Design review of the part built by this model. Coordinates are the model's own, in mm. Face numbers are marked on the shaded views. A direction names the side the tool comes from. Round coordinates to 2 decimals unless told otherwise and drop trailing zeros. Loops run counter-clockwise (first coordinate to the right, second up) from the corner with the lowest first, then second, coordinate; pieces in that order, holes last. Notation, with made-up numbers: (-26, 76) - (3, 76) arc R3 ccw to (3, 81) - close; hole circle Ø5 at (3, 60). An arc over 180 degrees is marked (long way). Use one line per item in the form item = value. Start each with the question number.
(1) We need section B-B, the plane z = 23. Write out the cut boundary in (x, y), then the cut area to 3 significant figures.
(2) Machinability: for the marked faces 1, 2 and 3, which of the approach directions +Z, -Z, +X, -X, +Y, -Y give a long, thin tool a straight path to every point of the face, cutting with its end or side? Answer none if there is none.
(3) We need section A-A, the plane z = 62.5. Write out the cut boundary in (x, y), then the cut area to 3 significant figures.
(4) We need section C-C, the plane z = 44. Write out the cut boundary in (x, y).
(5) For pin 1 (5.5 mm diameter, centred on x = -1, z = 48, fed in from -Y); pin 2 (2 mm diameter, centred on y = -5.5, z = 49.5, fed in from +X); pin 3 (3 mm diameter, centred on y = -5.5, z = 53, fed in from -X), all flat-tipped, find the tip position at first contact; note any pin that passes through.
(6) Wall thickness on probe 1 along Z at (x, y) = (2.75, -7.75); probe 2 along X at (y, z) = (0.5, 53); probe 3 along Z at (x, y) = (1.5, -4.25): over which ranges is each line inside the solid? List them lowest first. Write a range as [from, to].
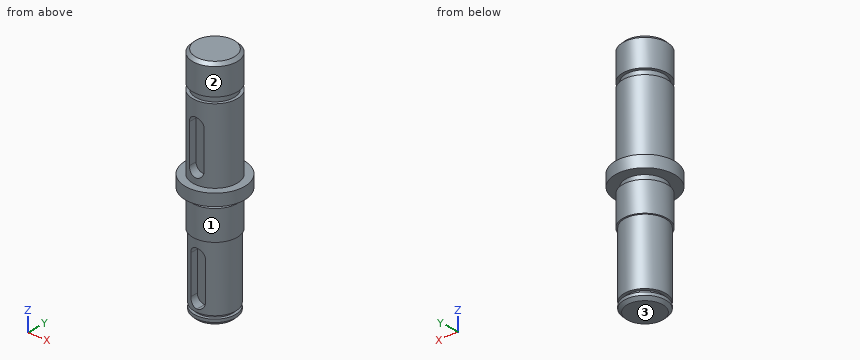
from build123d import *

# Parameters (mm, degrees)
SKETCH2_R           = 7
BOSS_EXTRUDE1_DEPTH = 2
SKETCH3_R           = 6
BOSS_EXTRUDE2_DEPTH = 1
SKETCH4_R           = 7
BOSS_EXTRUDE3_DEPTH = 22
SKETCH5_R           = 7.5
BOSS_EXTRUDE4_DEPTH = 10
SKETCH6_R           = 6.5
BOSS_EXTRUDE5_DEPTH = 2
SKETCH7_R           = 10
BOSS_EXTRUDE6_DEPTH = 4
SKETCH8_R           = 7.5
BOSS_EXTRUDE7_DEPTH = 25
SKETCH9_R           = 6.5
BOSS_EXTRUDE8_DEPTH = 2
SKETCH10_R          = 7.5
BOSS_EXTRUDE9_DEPTH = 10
CHAMFER1_SIZE       = 1
CUT_EXTRUDE1_START  = -4
CUT_EXTRUDE1_DEPTH  = 10
CUT_EXTRUDE2_START  = -4.5
CUT_EXTRUDE2_DEPTH  = 10


with BuildPart() as part:
    # Sketch2 → Boss-Extrude1 (new body)
    with BuildSketch(Plane.XY):
        Circle(SKETCH2_R)
    extrude(amount=BOSS_EXTRUDE1_DEPTH)

    # Sketch3 → Boss-Extrude2 (add)
    with BuildSketch(Plane.XY.offset(2)):
        Circle(SKETCH3_R)
    extrude(amount=BOSS_EXTRUDE2_DEPTH)

    # Sketch4 → Boss-Extrude3 (add)
    with BuildSketch(Plane.XY.offset(3)):
        Circle(SKETCH4_R)
    extrude(amount=BOSS_EXTRUDE3_DEPTH)

    # Sketch5 → Boss-Extrude4 (add)
    with BuildSketch(Plane.XY.offset(25)):
        Circle(SKETCH5_R)
    extrude(amount=BOSS_EXTRUDE4_DEPTH)

    # Sketch6 → Boss-Extrude5 (add)
    with BuildSketch(Plane.XY.offset(35)):
        Circle(SKETCH6_R)
    extrude(amount=BOSS_EXTRUDE5_DEPTH)

    # Sketch7 → Boss-Extrude6 (add)
    with BuildSketch(Plane.XY.offset(37)):
        Circle(SKETCH7_R)
    extrude(amount=BOSS_EXTRUDE6_DEPTH)

    # Sketch8 → Boss-Extrude7 (add)
    with BuildSketch(Plane.XY.offset(41)):
        Circle(SKETCH8_R)
    extrude(amount=BOSS_EXTRUDE7_DEPTH)

    # Sketch9 → Boss-Extrude8 (add)
    with BuildSketch(Plane.XY.offset(66)):
        Circle(SKETCH9_R)
    extrude(amount=BOSS_EXTRUDE8_DEPTH)

    # Sketch10 → Boss-Extrude9 (add)
    with BuildSketch(Plane.XY.offset(68)):
        Circle(SKETCH10_R)
    extrude(amount=BOSS_EXTRUDE9_DEPTH)

    # Chamfer1
    chamfer1_edges = [part.edges().sort_by_distance(p)[0] for p in [
        (-7, 0, 0),
        (-7.5, 0, 78),
    ]]
    chamfer(chamfer1_edges, length=CHAMFER1_SIZE)

    # Sketch11 → Cut-Extrude1 (cut)
    with BuildSketch(Plane(origin=(0, 0, 0), x_dir=(1, 0, 0), z_dir=(0, 1, 0)).offset(CUT_EXTRUDE1_START)):
        with BuildLine():
            ThreePointArc((2.5, -6.5), (1.767766953, -4.732233047), (0, -4))
            Line((0, -4), (0, -22))
            ThreePointArc((0, -22), (1.767766953, -21.267766953), (2.5, -19.5))
            Line((2.5, -19.5), (2.5, -6.5))
        make_face()
        with BuildLine():
            Line((0, -22), (0, -4))
            ThreePointArc((0, -4), (-1.767766953, -4.732233047), (-2.5, -6.5))
            Line((-2.5, -6.5), (-2.5, -19.5))
            ThreePointArc((-2.5, -19.5), (-1.767766953, -21.267766953), (0, -22))
        make_face()
    extrude(amount=-CUT_EXTRUDE1_DEPTH, mode=Mode.SUBTRACT)

    # Sketch12 → Cut-Extrude2 (cut)
    with BuildSketch(Plane(origin=(0, 0, 0), x_dir=(1, 0, 0), z_dir=(0, 1, 0)).offset(CUT_EXTRUDE2_START)):
        with BuildLine():
            Line((2.5, -45.5), (2.5, -58.5))
            ThreePointArc((2.5, -58.5), (0, -61), (-2.5, -58.5))
            Line((-2.5, -58.5), (-2.5, -45.5))
            ThreePointArc((-2.5, -45.5), (0, -43), (2.5, -45.5))
        make_face()
    extrude(amount=-CUT_EXTRUDE2_DEPTH, mode=Mode.SUBTRACT)


solid = part.part
Data:
q1.outline = circle Ø14 at (0, 0)
q1.area = 154 mm^2
q2.face_1 = -Z
q2.face_2 = +Z
q2.face_3 = -Z, +X, -X, +Y, -Y
q3.outline = circle Ø15 at (0, 0)
q3.area = 177 mm^2
q4.outline = (-2, -7.23) - (-2, -4.5) - (2, -4.5) - (2, -7.23) arc R7.5 ccw (long way) to start
q5.pin_1 = -7.07
q5.pin_2 = 6
q5.pin_3 = -6.34
q6.probe_1 = [37, 41]
q6.probe_2 = [-7.48, 7.48]
q6.probe_3 = [0, 4.5], [21.5, 78]
